Could you check a few things on this model? Use its own coordinates, in mm. A direction names the side the tool comes from. Coordinates: 2 decimals unless noted, no trailing zeros. Order: outer loops, then holes, each group sorted by start corner. A loop starts at its lowest first (then second) coordinate and runs counter-clockwise, first axis right, second up. Notation, with made-up numbers: (77.25, 50) -> (108.25, 50) arc R20 ccw to (108.25, 68) -> close; hole circle Ø8 at (11.5, 1.5). An arc over 180 degrees is marked (long way). Put each result on its own line as item: value. Start each with the question number.
Q1. If we section it at A-A (x = 0): Please give me the cut outline in (y, z), and give its area (3 significant figures).
Q2. If we section it at B-B (y = 0): Please give me the cut outline in (x, z), and give its area (3 significant figures).
Q3. If we section it at C-C (z = 13.25): Please give me the cut outline in (x, y).
Q4. Will these pins go through, and if not, where does the flat tip stop? pin 1 (5.5 mm diameter, centred on y = 29.5, z = 4, fed in from +X); pin 2 (5 mm diameter, centred on x = -4, y = -6.5, fed in from +Z); pin 3 (1 mm diameter, centred on y = -6, z = 13.5, fed in from +X); pin 4 (8 mm diameter, centred on x = -25, z = 12.5, fed in from -Y).
Q5. If we section it at D-D (z = 4.75): Please give me the cut outline in (x, y).
Q6. For faces 1 (the face through (-0.16, 31.77, 14.45)), 2 (the face through (1.223, -28.974, 1.704)), 3 (the face through (0.1, 32.1, 9.4)), which set-ups out of +Z, -Z, +X, -X, +Y, -Y let a thin tool reach every point of the face, with its end or its side?
Q7. Please list where these lines run through material, in increasing order: line 1 along Z through (x, y) = (0, 12); line 2 along X through (y, z) = (0, 1.9); line 3 along Y through (x, z) = (20, 9.5).
from build123d import *

# Parameters (mm, degrees)
SKETCH_1_R           = 35.9
EXTRUDE_1_DEPTH      = 19
EXTRUDE_1_TAPER      = 40
EXTRUDE_2_DEPTH      = 40
EXTRUDE_3_REACH      = 59.007
SKETCH_8_R           = 31
SKETCH_8_R_2         = 29
SKETCH_9_R           = 8.8
CUT_EXTRUDE_1_DEPTH  = 2
CUT_EXTRUDE_2_DEPTH  = 16
EXTRUDE_4_REACH      = 88.085
EXTRUDE_4_END_RADIUS = 31
SKETCH_11_W          = 2.2
SKETCH_11_H          = 6.7


with BuildPart() as part:
    # 草图1 → 凸台-拉伸1 (new body)
    with BuildSketch(Plane.XY):
        Circle(SKETCH_1_R)
    extrude(amount=EXTRUDE_1_DEPTH, taper=EXTRUDE_1_TAPER)

    # 草图6 → 凸台-拉伸2 (add)
    with BuildSketch(Plane(origin=(0, 0, 0), x_dir=(1, 0, 0), z_dir=(0, 1, 0))):
        with BuildLine():
            Line((-7.2, 0), (-7.2, -7.25))
            ThreePointArc((-7.2, -7.25), (0, -14.45), (7.2, -7.25))
            Line((7.2, -7.25), (7.2, 0))
            Line((7.2, 0), (-7.2, 0))
        make_face()
    extrude(amount=EXTRUDE_2_DEPTH)

    # 草图7 → 切除-旋转1 (revolve, cut)
    with BuildSketch(Plane(origin=(0, 0, 0), x_dir=(0, 0, -1), z_dir=(1, 0, 0)), mode=Mode.PRIVATE) as cut_revolve_1_sk:
        Polygon((-17, 0), (-17, -17.63530627), (0, -31.9), (0, 0), align=None)
    revolve(cut_revolve_1_sk.sketch.rotate(Axis((0, 0, -9.48864884), (0, 0, 1)), 270), axis=Axis((0, 0, -9.48864884), (0, 0, 1)), mode=Mode.SUBTRACT)

    # 凸台-拉伸3: up to this cone (the profile starts inside it)
    extrude_3_end = Plane(origin=(0, 0, 0), z_dir=(0, 0, -1)).offset(-38.016938604) * Cone(1e-06, 108.599579987, 129.423938604, align=(Align.CENTER, Align.CENTER, Align.MIN), mode=Mode.PRIVATE)
    # 草图8 → 凸台-拉伸3 (add, up to the surface)
    with BuildSketch(Plane(origin=(0, 0, 0), x_dir=(-1, 0, 0), z_dir=(0, 0, -1)), mode=Mode.PRIVATE) as extrude_3_sk1:
        Circle(SKETCH_8_R)
        Circle(SKETCH_8_R_2, mode=Mode.SUBTRACT)
    extrude_3_tool1 = extrude(extrude_3_sk1.sketch, amount=-EXTRUDE_3_REACH, mode=Mode.PRIVATE) & extrude_3_end
    add(extrude_3_tool1.solids().sort_by_distance((30.123188, 0, 0))[0])

    # 草图9 → 切除-拉伸1 (cut)
    with BuildSketch(Plane.XY.offset(19)):
        Circle(SKETCH_9_R)
    extrude(amount=-CUT_EXTRUDE_1_DEPTH, mode=Mode.SUBTRACT)

    # 草图10 → 切除-拉伸2 (cut)
    with BuildSketch(Plane(origin=(0, 40, 0), x_dir=(1, 0, 0), z_dir=(0, 1, 0))):
        with BuildLine():
            Line((3.7, 0), (3.7, -6.7))
            Line((3.7, -6.7), (2.7, -6.7))
            ThreePointArc((2.7, -6.7), (0, -9.4), (-2.7, -6.7))
            Line((-2.7, -6.7), (-3.7, -6.7))
            Line((-3.7, -6.7), (-3.7, 0))
            Line((-3.7, 0), (3.7, 0))
        make_face()
    extrude(amount=-CUT_EXTRUDE_2_DEPTH, mode=Mode.SUBTRACT)

    # 凸台-拉伸4: up to this cylinder (the profile starts outside it)
    extrude_4_end = Plane(origin=(0, 0, 3.35), z_dir=(0, 0, -1)) * Cylinder(EXTRUDE_4_END_RADIUS, 239.17, mode=Mode.PRIVATE)
    # 草图11 → 凸台-拉伸4 (add, up to the surface)
    with BuildSketch(Plane(origin=(0, 40, 0), x_dir=(1, 0, 0), z_dir=(0, 1, 0)), mode=Mode.PRIVATE) as extrude_4_sk1:
        with Locations((-4.8, -3.35)):
            Rectangle(SKETCH_11_W, SKETCH_11_H)
    extrude_4_tool1 = extrude(extrude_4_sk1.sketch, amount=-EXTRUDE_4_REACH, mode=Mode.PRIVATE) - extrude_4_end
    add(extrude_4_tool1.solids().sort_by_distance((-4.8, 40, 3.35))[0])
    # 草图11 → 凸台-拉伸4 (add, up to the surface)
    with BuildSketch(Plane(origin=(0, 40, 0), x_dir=(1, 0, 0), z_dir=(0, 1, 0)), mode=Mode.PRIVATE) as extrude_4_sk2:
        with Locations((4.8, -3.35)):
            Rectangle(SKETCH_11_W, SKETCH_11_H)
    extrude_4_tool2 = extrude(extrude_4_sk2.sketch, amount=-EXTRUDE_4_REACH, mode=Mode.PRIVATE) - extrude_4_end
    add(extrude_4_tool2.solids().sort_by_distance((4.8, 40, 3.35))[0])


solid = part.part
The answers:
1. outline: (-35.9, 0) -> (-31.9, 0) -> (-31, 1.07) -> (-31, 0) -> (-29, 0) -> (-29, 3.46) -> (-17.64, 17) -> (-8.8, 17) -> (-8.8, 19) -> (-19.96, 19) -> close; (8.8, 17) -> (17.64, 17) -> (24.01, 9.4) -> (40, 9.4) -> (40, 14.45) -> (23.78, 14.45) -> (19.96, 19) -> (8.8, 19) -> close
1. area: 222 mm^2
2. outline: (-35.9, 0) -> (-31.9, 0) -> (-31, 1.07) -> (-31, 0) -> (-29, 0) -> (-29, 3.46) -> (-17.64, 17) -> (-8.8, 17) -> (-8.8, 19) -> (-19.96, 19) -> close; (8.8, 17) -> (17.64, 17) -> (29, 3.46) -> (29, 0) -> (31, 0) -> (31, 1.07) -> (31.9, 0) -> (35.9, 0) -> (19.96, 19) -> (8.8, 19) -> close
2. area: 193 mm^2
3. outline: (-3.98, 24.46) arc R24.78 ccw (long way) to (3.98, 24.46) -> (3.98, 40) -> (-3.98, 40) -> close; hole circle Ø41.56 at (0, 0)
4. pin 1: x = 20.22
4. pin 2: z = 19
4. pin 3: x = 24.28
4. pin 4: y = -16.75
5. outline: (-7.2, 31.09) arc R31.91 ccw (long way) to (7.2, 31.09) -> (7.2, 40) -> (3.7, 40) -> (3.7, 27.67) arc R27.91 cw (long way) to (-3.7, 27.67) -> (-3.7, 40) -> (-7.2, 40) -> close
6. face 1: +Z, +Y
6. face 2: -Z
6. face 3: -Z, +Y
7. line 1: 17 to 19
7. line 2: -34.31 to -29, 29 to 34.31
7. line 3: -19.49 to -13.14, 13.14 to 19.49
